from build123d import *

# Parameters (mm, degrees)
PEDESTAL_BODY_DEPTH  = 100
FRONT_BOSS_DEPTH     = 35
FRONT_BOSS_CUT_DEPTH = 359.742254771
TOP_BOSS_DEPTH       = 35
TOP_BOSS_CUT_A_DEPTH = 324.745166661
TOP_BOSS_CUT_B_DEPTH = 339.016839686


with BuildPart() as part:
    # Pedestal Profile Sketch → Pedestal Body (new, symmetric)
    with BuildSketch(Plane.XY):
        Polygon((40, 0), (40, 60), (-40, 60), (-40, 0), (-150, 0), (-80, 253.467957262), (-25, 253.467957262), (-25, 217.876631195), (25, 217.876631195), (25, 253.467957262), (80, 253.467957262), (150, 0), align=None)
    extrude(amount=PEDESTAL_BODY_DEPTH, both=True)

    # Front Boss Sketch → Front Boss (add)
    with BuildSketch(Plane.XY.offset(100)):
        Polygon((40, 0), (65, 0), (65, 130), (-65, 130), (-65, 0), (-40, 0), (-40, 60), (40, 60), align=None)
    extrude(amount=FRONT_BOSS_DEPTH)

    # Front Boss Cut Sketch → Front Boss Cut (cut, through all)
    with BuildSketch(Plane.ZY.offset(65)):
        Polygon((100, 0), (135, 130), (135, 0), align=None)
    extrude(amount=-FRONT_BOSS_CUT_DEPTH, mode=Mode.SUBTRACT)

    # Top Boss Sketch → Top Boss (add)
    with BuildSketch(Plane(origin=(-139.370318702, 38.489765785, 0), x_dir=(0, 0, 1), z_dir=(-0.9639167277376053, 0.26620394810676146, 0))):
        Polygon((-100, -39.930592216), (0, 70.069407784), (100, -39.930592216), align=None)
    extrude(amount=TOP_BOSS_DEPTH)

    # Top Boss Cut A Sketch → Top Boss Cut A (cut, through all)
    with BuildSketch(Plane(origin=(8.440159726, 30.561572066, 34.87617582), x_dir=(0.9838366716003674, -0.11801541262610508, -0.13467652355552237), z_dir=(0.1790681535458246, 0.6484005584270376, 0.7399400733959439))):
        Polygon((-161.043153096, -65.90530493), (-165.570989176, 86.752805567), (-195.334500882, -58.897918327), align=None)
    extrude(amount=-TOP_BOSS_CUT_A_DEPTH, mode=Mode.SUBTRACT)

    # Top Boss Cut B Sketch → Top Boss Cut B (cut, through all)
    with BuildSketch(Plane(origin=(8.440159726, 30.561572066, -34.87617582), x_dir=(-0.9838366716003674, 0.11801541262610508, -0.13467652355552237), z_dir=(0.1790681535458246, 0.6484005584270376, -0.7399400733959439))):
        Polygon((161.043153096, -65.90530493), (165.570989176, 86.752805567), (192.07604702, -59.563778593), align=None)
    extrude(amount=-TOP_BOSS_CUT_B_DEPTH, mode=Mode.SUBTRACT)


solid = part.part
Check sheet for the modelled part. Datum: model origin and axes. Units: mm. A direction names the side the tool comes from. Give positions to 0.01 mm unless a question says otherwise; leave off trailing zeros. Write each loop counter-clockwise with the first axis right and the second up, starting at its lowest first coordinate (ties: lowest second). Pieces come first, ordered by that corner, then holes. Notation, with made-up numbers: (-25, 22) -> (-10, 22) arc R21 ccw to (-10, 46) -> close; hole circle Ø6 at (76, -11). An arc over 180 degrees is marked (long way). Use one line per item in the form item = value. Start each with the question number.
1. Mould release check, pull along X, two halves, no side actions. Record for faces 6 (the flat face through (-157.256, 38.544, -29.791)), 7 (the flat face through (-40, 30, 7)), 8 (the flat face through (2, 157, 100)), 9 (the flat face through (-138.192, 78.358, -28.478)): pulls with the +X half, pulls with the -X half, needs draft (parallel to the pull), parting line crosses it, or undercut.
2. Section check A-A (y = 16.5). Record the cut outline in (x, z), and give its area (3 significant figures).
3. Access from +Z, -Z, +X, -X, +Y, -Y to the whole of each face (thin tool, end or side, straight path). Record for faces 1 (the flat face through (65, 93, 109)), 2 (the flat face through (-65, 80, 113)), 3 (the flat face through (1, 130, 117)), 4 (the flat face through (-144.784, 69.097, 38.189)), 5 (the flat face through (40, 30, 7)).
4. Section check C-C (z = -76). Record the cut outline in (x, y), and give its area (3 significant figures).
5. Section check B-B (x = -50). Record the cut outline in (y, z), and give its area (3 significant figures).
6. Thickness scan on line 1 along X through (y, z) = (56, 115); line 2 along Y through (x, z) = (-1.5, 40); line 3 along Z through (x, y) = (91.5, 12.5). Record the ranges inside material, lowest first. Write a range as from..to.
7. Section check D-D (y = 123). Record the cut outline in (x, z), and give its area (3 significant figures).
8. Go/stop test with flat-tipped pins: P1, Ø3, axis at y = 86.5, z = 26.5, coming from the +X side; P2, Ø1.5, axis at y = 32.5, z = -68.5, coming from the -X side; P3, Ø25, axis at x = 2.5, z = -42.5, coming from the +Y side; P4, Ø8, axis at x = 91, z = 43, coming from the -Y side. Record where each tip stops, or that it passes through.
Conclusion:
q1.face_6 = pulls with the -X half
q1.face_7 = undercut
q1.face_8 = needs draft
q1.face_9 = undercut
q2.outline = (-164.07, 0) -> (-150.64, -85.7) -> (-145.44, -84.44) -> (-145.44, -100) -> (-40, -100) -> (-40, 104.44) -> (-65, 104.44) -> (-65, 100) -> (-145.44, 100) -> (-145.44, 84.44) -> (-150.64, 85.7) -> close; (40, -100) -> (145.44, -100) -> (145.44, 100) -> (65, 100) -> (65, 104.44) -> (40, 104.44) -> close
q2.area = 44,400 mm²
q3.face_1 = +Z, +X, +Y, -Y
q3.face_2 = +Z, -X, +Y, -Y
q3.face_3 = +Z, +X, -X, +Y
q3.face_4 = +Z, +Y
q3.face_5 = +Z, -Z, -Y
q4.outline = (-153.66, 1.01) -> (-150, 0) -> (-40, 0) -> (-40, 60) -> (40, 60) -> (40, 0) -> (150, 0) -> (80, 253.47) -> (25, 253.47) -> (25, 217.88) -> (-25, 217.88) -> (-25, 253.47) -> (-80, 253.47) -> (-142.97, 25.45) -> (-151.07, 27.68) -> close
q4.area = 51,900 mm²
q5.outline = (0, -100) -> (253.47, -100) -> (253.47, 100) -> (130, 100) -> (130, 135) -> (0, 100) -> close
q5.area = 53,000 mm²
q6.line_1 = -65..-40, 40..65
q6.line_2 = 60..217.88
q6.line_3 = -100..100
q7.outline = (-116.03, -100) -> (116.03, -100) -> (116.03, 100) -> (65, 100) -> (65, 133.12) -> (-65, 133.12) -> (-65, 100) -> (-116.03, 100) -> close
q7.area = 50,700 mm²
q8.P1 = 126.53
q8.P2 = -151.91
q8.P3 = 217.88
q8.P4 = 0
